The listing builds one solid part. Answer for the finished solid, in the listing's coordinates (mm). Give positions to 0.01 mm unless a question says otherwise; leave off trailing zeros. Order: outer loops, then holes, each group sorted by start corner. A loop starts at its lowest first (then second) coordinate and runs counter-clockwise, first axis right, second up. Notation, with made-up numbers: (4, 84) - (38, 84) arc R23 ccw to (38, 109) - close; hole circle Ø4 at (37, 55). An arc over 180 degrees is marked (long way). Answer as a JSON object with one key per item and string values. Group by question number.
Q1. Consider line 1 (X direction, y = 68.5, z = -1.9); line 2 (X direction, y = 82.5, z = 1.1). Determine where each line is inside the solid, lowest interval first.
Q2. A cutting plane is placed at B-B, the plane x = 31. Give the vertices of the cut face in (y, z).
Q3. A cutting plane is placed at C-C, the plane y = 102.5. Give the vertices of the cut face in (x, z), and give its area (3 significant figures).
Q4. A cutting plane is placed at A-A, the plane z = 0.1. Give the vertices of the cut face in (x, y), and give its area (4 significant figures).
from build123d import *

# Parameters (mm, degrees)
EXTRUDE_1_DEPTH = 2.5


with BuildPart() as part:
    # 草图1 → 凸台-拉伸1 (new, symmetric)
    with BuildSketch(Plane.XY):
        Polygon((0, 0), (0, 150), (20, 150), (45, 20), (45, 0), align=None)
    extrude(amount=EXTRUDE_1_DEPTH, both=True)


solid = part.part
Reply:
{
 "1": {"line 1": "x = 0 to 35.67", "line 2": "x = 0 to 32.98"},
 "2": {"outline": "(0, -2.5) - (92.8, -2.5) - (92.8, 2.5) - (0, 2.5) - close"},
 "3": {"outline": "(0, -2.5) - (29.13, -2.5) - (29.13, 2.5) - (0, 2.5) - close", "area": "146 mm^2"},
 "4": {"outline": "(0, 0) - (45, 0) - (45, 20) - (20, 150) - (0, 150) - close", "area": "5,125 mm^2"}
}
